Verification items for this drawing (mm, ordinates from the low corner). A direction names the side the tool comes from. Round coordinates to 2 decimals unless told otherwise and drop trailing zeros. Order: outer loops, then holes, each group sorted by start corner. A loop starts at its lowest first (then second) coordinate and runs counter-clockwise, first axis right, second up. Notation, with made-up numbers: M 32.5,-3 L 66.5,-3 A20 ccw 66.5,21 Z; hole C 61.5,45 d8. An arc over 180 degrees is marked long. Use CSV: the item, a comma, the result in double quotes. Start each with the question number.
Q1. Gauge pin test, flat ends, axial feed: pin 1 Ø4 at (x, y) = (31.5, 6.5) entering from -Z; pin 2 Ø3 at (x, z) = (65.5, 10) entering from -Y; pin 3 Ø3 at (x, y) = (29, 8.5) entering from +Z; pin 4 Ø1.5 at (y, z) = (5.5, 2) entering from +X. Record the tip position at first contact, or that the pin passes through.
Q2. Sectioned sample at B-B (z = 6). Enter the section's corners in (x, y).
Q3. Sectioned sample at C-C (x = 5). Enter the section's corners in (y, z), and give its area (3 significant figures).
Q4. Set-up check for the marked faces 1 and 2: record each of +Z, -Z, +X, -X, +Y, -Y from which the full face is reachable in a straight line by a thin tool's end or side.
Q5. Sectioned sample at A-A (y = 6). Enter the section's corners in (x, z), and give its area (3 significant figures).
Q6. Scan lines: line 1 (X direction, y = 7.75, z = 1); line 2 (X direction, y = 2.25, z = 2); line 3 (Y direction, x = 5, z = 5.75). Record each from-to range of solid material in increasing order.
Q7. Sectioned sample at D-D (x = 45). Enter the section's corners in (y, z), and give its area (3 significant figures).
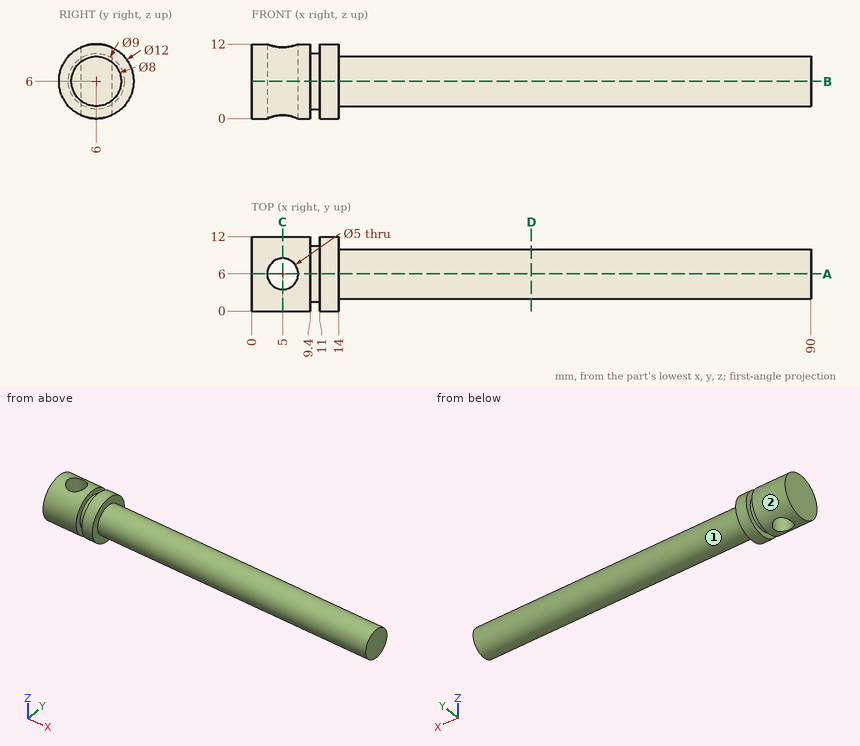
Verdict:
1,pin 1,"stops at z = 2"
1,pin 2,"stops at y = 2.88"
1,pin 3,"stops at z = 9.87"
1,pin 4,"stops at x = 90"
2,outline,"M 0,0 L 9.4,0 L 9.4,1.5 L 11,1.5 L 11,0 L 14,0 L 14,2 L 90,2 L 90,10 L 14,10 L 14,12 L 11,12 L 11,10.5 L 9.4,10.5 L 9.4,12 L 0,12 Z; hole C 5,6 d5"
3,outline,"M 3.5,0.55 L 3.5,11.45 A6 ccw Z; M 8.5,0.55 A6 ccw 8.5,11.45 Z"
3,area,"54.9 mm²"
4,face 1,"+X"
4,face 2,"+X, -X"
5,outline,"M 0,0 L 2.5,0 L 2.5,12 L 0,12 Z; M 7.5,0 L 9.4,0 L 9.4,1.5 L 11,1.5 L 11,0 L 14,0 L 14,2 L 90,2 L 90,10 L 14,10 L 14,12 L 11,12 L 11,10.5 L 9.4,10.5 L 9.4,12 L 7.5,12 Z"
5,area,"711 mm²"
6,line 1,"x = 0 to 3.21, 6.79 to 9.4, 11 to 14"
6,line 2,"x = 0 to 9.4, 11 to 14"
6,line 3,"y = 0.01 to 3.5, 8.5 to 11.99"
7,outline,"C 6,6 d8"
7,area,"50.3 mm²"
